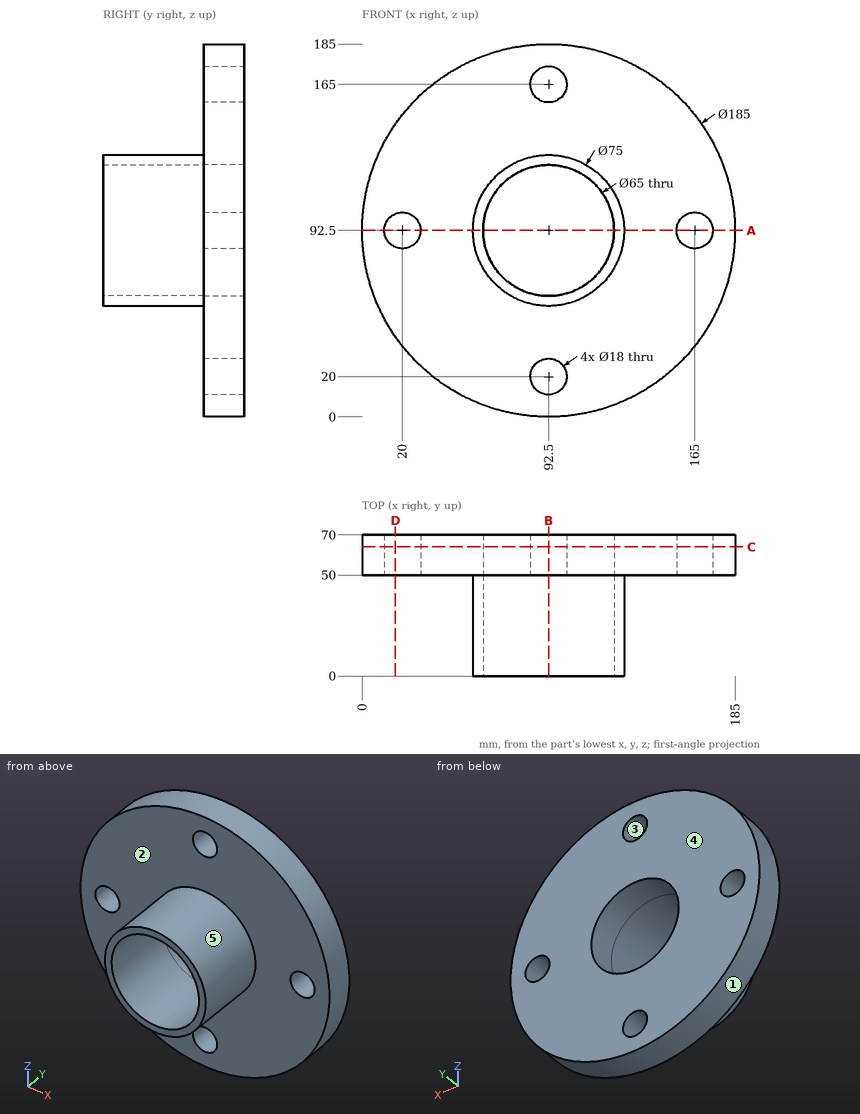
Design review of the part shown in the three views and the two pictorial views. Dimensions are in mm from the part's minimum x, y and z. A direction names the side the tool comes from. Coordinates: 2 decimals unless noted, no trailing zeros. Write each loop counter-clockwise with the first axis right and the second up, starting at its lowest first coordinate (ties: lowest second). Pieces come first, ordered by that corner, then holes. Notation, with made-up numbers: (-11.5, 3.5) -> (-1.5, 3.5) arc R24 cw to (-1.5, 37.5) -> close; hole circle Ø4 at (19, 0.5). An arc over 180 degrees is marked (long way). Answer in a Markdown table with one row per item.
1. Wall thickness on probe 1 along Z at (x, y) = (92, 64); probe 2 along X at (y, z) = (19, 92); probe 3 along X at (y, z) = (55.5, 92.5): over which ranges is each line inside the solid? List them lowest first. Write a range as [from, to].
Answers below:
| item | result |
|---|---|
| probe 1 | z = [0, 11.01], [28.99, 60], [125, 156.01], [173.99, 185] |
| probe 2 | x = [55, 60], [125, 130] |
| probe 3 | x = [0, 11], [29, 60], [125, 156], [174, 185] |
2. Clearance check with flat-ended pins moving along their axes: pin 1 Ø2 at (x, y) = (124.5, 25.5) entering from -Z; pin 2 Ø3 at (y, z) = (29, 78) entering from -X; pin 3 Ø1.5 at (y, z) = (16, 67) entering from +X. State where each tip first meets the part, or that it passes through.
Answers below:
| item | result |
|---|---|
| pin 1 | stops at z = 71.4 |
| pin 2 | stops at x = 57.33 |
| pin 3 | stops at x = 120.67 |
3. We need section C-C, the plane y = 64. State the section outline as (x, z) points.
Answers below:
| item | result |
|---|---|
| outline | circle Ø185 at (92.5, 92.5); hole circle Ø18 at (20, 92.5); hole circle Ø65 at (92.5, 92.5); hole circle Ø18 at (92.5, 20); hole circle Ø18 at (92.5, 165); hole circle Ø18 at (165, 92.5) |
4. We need section D-D, the plane x = 16.5. State the section outline as (y, z) points.
Answers below:
| item | result |
|---|---|
| outline | (50, 39.77) -> (70, 39.77) -> (70, 84.21) -> (50, 84.21) -> close; (50, 100.79) -> (70, 100.79) -> (70, 145.23) -> (50, 145.23) -> close |
5. Draft analysis for pull direction X (two halves, no side actions). For the marked faces 1, 2 and 3, state which applies: +X half, -X half, draft (parallel to the pull), parting line (faces both ways), or undercut.
Answers below:
| item | result |
|---|---|
| face 1 | parting line |
| face 2 | draft |
| face 3 | undercut |
6. For the marked faces 4 and 5, list the 3-axis set-ups (+Z, -Z, +X, -X, +Y, -Y) from which the entire face can be reached by the end or side of a thin tool; tool diameter is ignored.
Answers below:
| item | result |
|---|---|
| face 4 | +Z, -Z, +X, -X, +Y |
| face 5 | -Y |
7. We need section B-B, the plane x = 92.5. State the section outline as (y, z) points, and give its area (3 significant figures).
Answers below:
| item | result |
|---|---|
| outline | (0, 55) -> (50, 55) -> (50, 29) -> (70, 29) -> (70, 60) -> (0, 60) -> close; (0, 125) -> (70, 125) -> (70, 156) -> (50, 156) -> (50, 130) -> (0, 130) -> close; (50, 0) -> (70, 0) -> (70, 11) -> (50, 11) -> close; (50, 174) -> (70, 174) -> (70, 185) -> (50, 185) -> close |
| area | 2,180 mm^2 |
8. We need section A-A, the plane z = 92.5. State the section outline as (x, y) points.
Answers below:
| item | result |
|---|---|
| outline | (0, 50) -> (11, 50) -> (11, 70) -> (0, 70) -> close; (29, 50) -> (55, 50) -> (55, 0) -> (60, 0) -> (60, 70) -> (29, 70) -> close; (125, 0) -> (130, 0) -> (130, 50) -> (156, 50) -> (156, 70) -> (125, 70) -> close; (174, 50) -> (185, 50) -> (185, 70) -> (174, 70) -> close |
